Here's the drawing with two shaded views (mm, measured from the low corner). I have some questions. A direction names the side the tool comes from. Give positions to 0.01 mm unless a question says otherwise; leave off trailing zeros. Write each loop counter-clockwise with the first axis right and the second up, starting at its lowest first coordinate (ties: lowest second). Pieces come first, ordered by that corner, then holes. Notation, with made-up numbers: (60, 12.25) -> (92, 12.25) arc R23 ccw to (92, 23.25) -> close; hole circle Ø4 at (-37, 20.5). An arc over 180 degrees is marked (long way). One line per item, written item: value.
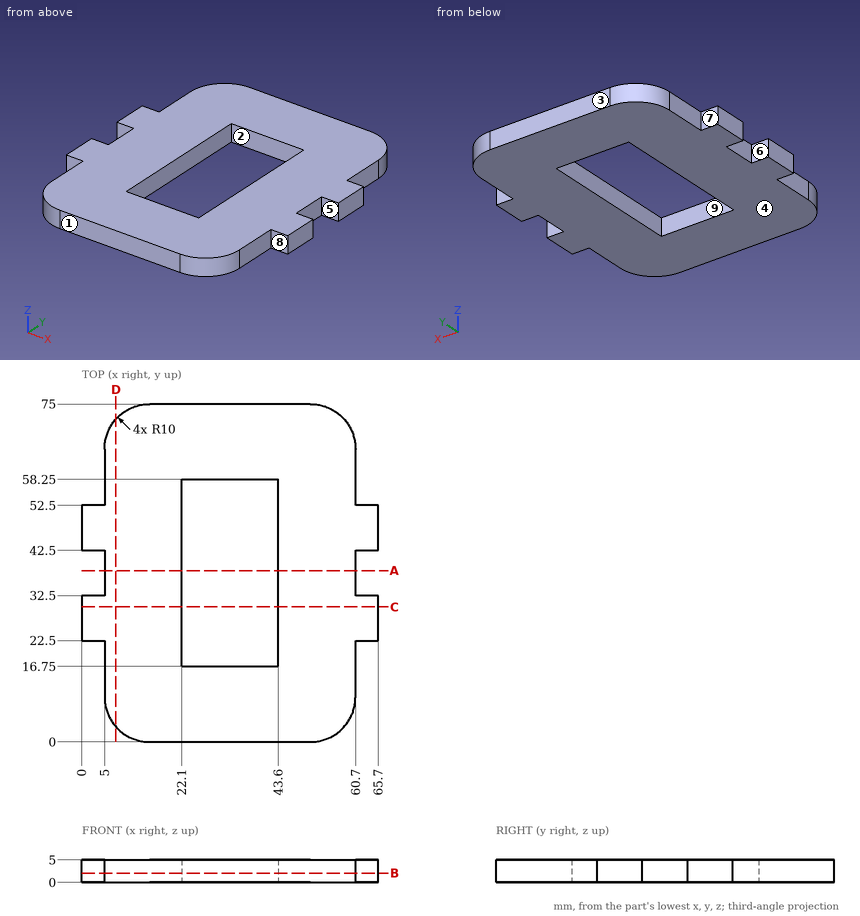
1) If we section it at D-D (x = 7.5): Write out the boundary of the cut face in (y, z), and give its area (3 significant figures).
Answer list:
outline: (3.39, 0) -> (71.61, 0) -> (71.61, 5) -> (3.39, 5) -> close
area: 341 mm^2
2) For the marked faces 5, 6, 7, 8 and 9, which set-ups out of +Z, -Z, +X, -X, +Y, -Y let a thin tool reach every point of the face, with its end or its side?
Answer list:
face 5: +Z, -Z, +X
face 6: +Z, -Z, -X
face 7: +Z, -Z, -X, +Y
face 8: +Z, -Z, +X, -Y
face 9: +Z, -Z
3) We'd pull the mould along Y, two halves only. Please class the marked faces 1, 2, 3 and 4: released by +Y, released by -Y, zero draft, split by the parting line, or undercut.
Answer list:
face 1: released by -Y
face 2: undercut
face 3: released by +Y
face 4: zero draft
4) Will these pins go through, and if not, where does the flat tip stop? pin 1 (2.5 mm diameter, centred on x = 1.5, z = 3.5, fed in from +Y); pin 2 (2.5 mm diameter, centred on y = 36.5, z = 2, fed in from -X); pin 3 (2.5 mm diameter, centred on x = 1.5, z = 3.5, fed in from -Y).
Answer list:
pin 1: stops at y = 52.5
pin 2: stops at x = 5
pin 3: stops at y = 22.5
5) I need wall thicknesses on L1, parallel to Y at x = 35.5, z = 4.35; L2, parallel to X at y = 29.5, z = 0.8; L3, parallel to X at y = 21.5, z = 2.2. Which ranges of each line are inside material? Lowest first, please.
Answer list:
L1: y = 0 to 16.75, 58.25 to 75
L2: x = 0 to 22.1, 43.6 to 65.7
L3: x = 5 to 22.1, 43.6 to 60.7
6) If we section it at C-C (y = 30): Write out the boundary of the cut face in (x, z).
Answer list:
outline: (0, 0) -> (22.1, 0) -> (22.1, 5) -> (0, 5) -> close; (43.6, 0) -> (65.7, 0) -> (65.7, 5) -> (43.6, 5) -> close
7) If we section it at B-B (z = 2.05): Write out the boundary of the cut face in (x, y), and give its area (3 significant figures).
Answer list:
outline: (0, 22.5) -> (5, 22.5) -> (5, 10) arc R10 ccw to (15, 0) -> (50.7, 0) arc R10 ccw to (60.7, 10) -> (60.7, 22.5) -> (65.7, 22.5) -> (65.7, 32.5) -> (60.7, 32.5) -> (60.7, 42.5) -> (65.7, 42.5) -> (65.7, 52.5) -> (60.7, 52.5) -> (60.7, 65) arc R10 ccw to (50.7, 75) -> (15, 75) arc R10 ccw to (5, 65) -> (5, 52.5) -> (0, 52.5) -> (0, 42.5) -> (5, 42.5) -> (5, 32.5) -> (0, 32.5) -> close; hole (22.1, 16.75) -> (43.6, 16.75) -> (43.6, 58.25) -> (22.1, 58.25) -> close
area: 3,400 mm^2
8) If we section it at A-A (y = 38): Write out the boundary of the cut face in (x, z), and give its area (3 significant figures).
Answer list:
outline: (5, 0) -> (22.1, 0) -> (22.1, 5) -> (5, 5) -> close; (43.6, 0) -> (60.7, 0) -> (60.7, 5) -> (43.6, 5) -> close
area: 171 mm^2
